Part model, mm, in its own coordinate system. A direction names the side the tool comes from. Round coordinates to 2 decimals unless told otherwise and drop trailing zeros. Loops run counter-clockwise (first coordinate to the right, second up) from the corner with the lowest first, then second, coordinate; pieces in that order, holes last. Notation, with made-up numbers: M 76.5,84 L 109.5,84 A12 ccw 109.5,102 Z; hole C 74.5,56.5 d2. An arc over 180 degrees is marked long. Put each result on its own line as item: value. Start each with the question number.
```python
from build123d import *

# Parameters (mm, degrees)
GBT706_2008_16A_1_DEPTH = 1637
CUT_EXTRUDE_1_DEPTH     = 837.367891541
CUT_EXTRUDE_2_DEPTH     = 837.367891541
SKETCH_4_W              = 56.5
SKETCH_4_H              = 56.5
CUT_EXTRUDE_3_DEPTH     = 835.965313439
SKETCH_5_W              = 56.5
SKETCH_5_H              = 56.5
CUT_EXTRUDE_4_DEPTH     = 835.965313439
CUT_EXTRUDE_5_REACH     = 838.368


with BuildPart() as part:
    # Sketch12 → Gbt706-2008 热轧槽钢 16A(1) (new body)
    with BuildSketch(Plane.YZ.offset(-818.5)):
        with BuildLine():
            Line((63, 160), (0, 160))
            Line((0, 160), (0, 0))
            Line((0, 0), (63, 0))
            Line((63, 0), (63, 2.528785132))
            ThreePointArc((63, 2.528785132), (61.715724127, 5.874438164), (58.522642316, 7.501394609))
            Line((58.522642316, 7.501394609), (15.454715367, 12.028016136))
            ThreePointArc((15.454715367, 12.028016136), (9.068551745, 15.281929026), (6.5, 21.973235089))
            Line((6.5, 21.973235089), (6.5, 138.026764911))
            ThreePointArc((6.5, 138.026764911), (9.068551745, 144.718070974), (15.454715367, 147.971983864))
            Line((15.454715367, 147.971983864), (58.522642316, 152.498605391))
            ThreePointArc((58.522642316, 152.498605391), (61.715724127, 154.125561836), (63, 157.471214868))
            Line((63, 157.471214868), (63, 160))
        make_face()
    extrude(amount=GBT706_2008_16A_1_DEPTH)

    # 草图2 → 切除-拉伸1 (cut, through all)
    with BuildSketch(Plane.XZ):
        Polygon((762, -5), (762, 7.501394609), (766.477357684, 7.501394609), (809.545284633, 12.028016136), (818.5, 21.973235089), (818.5, 138.026764911), (809.545284633, 147.971983864), (766.477357684, 152.498605391), (762, 152.498605391), (762, 165), (828.5, 165), (828.5, -5), align=None)
    extrude(amount=-CUT_EXTRUDE_1_DEPTH, mode=Mode.SUBTRACT)

    # 草图3 → 切除-拉伸2 (cut, through all)
    with BuildSketch(Plane.XZ):
        Polygon((-762, 0), (-762, 7.501394609), (-766.477357684, 7.501394609), (-809.545284633, 12.028016136), (-818.5, 21.973235089), (-818.5, 138.026764911), (-809.545284633, 147.971983864), (-766.477357684, 152.498605391), (-762, 152.498605391), (-762, 165), (-838.5, 165), (-838.5, -5), (-762, -5), align=None)
    extrude(amount=-CUT_EXTRUDE_2_DEPTH, mode=Mode.SUBTRACT)

    # 草图4 → 切除-拉伸3 (cut, through all)
    with BuildSketch(Plane.XY.offset(152.498605391)):
        with Locations((790.25, 34.75)):
            Rectangle(SKETCH_4_W, SKETCH_4_H)
    extrude(amount=-CUT_EXTRUDE_3_DEPTH, mode=Mode.SUBTRACT)

    # 草图5 → 切除-拉伸4 (cut, through all)
    with BuildSketch(Plane.XY.offset(152.498605391)):
        with Locations((-790.25, 34.75)):
            Rectangle(SKETCH_5_W, SKETCH_5_H)
    extrude(amount=-CUT_EXTRUDE_4_DEPTH, mode=Mode.SUBTRACT)

    # 草图6 → 切除-拉伸5 (cut, up to next)
    with BuildSketch(Plane.XZ, mode=Mode.PRIVATE) as cut_extrude_5_sk1:
        with BuildLine():
            Line((-580, 20), (-720, 20))
            ThreePointArc((-720, 20), (-723.535533906, 21.464466094), (-725, 25))
            Line((-725, 25), (-725, 105))
            ThreePointArc((-725, 105), (-723.535533906, 108.535533906), (-720, 110))
            Line((-720, 110), (-580, 110))
            ThreePointArc((-580, 110), (-576.464466094, 108.535533906), (-575, 105))
            Line((-575, 105), (-575, 25))
            ThreePointArc((-575, 25), (-576.464466094, 21.464466094), (-580, 20))
        make_face()
    cut_extrude_5_tool1 = extrude(cut_extrude_5_sk1.sketch, amount=-CUT_EXTRUDE_5_REACH, mode=Mode.PRIVATE) & part.part
    # 草图6 → 切除-拉伸5 (cut, up to next)
    with BuildSketch(Plane.XZ, mode=Mode.PRIVATE) as cut_extrude_5_sk2:
        with BuildLine():
            Line((-375, 25), (-375, 105))
            ThreePointArc((-375, 105), (-376.464466094, 108.535533906), (-380, 110))
            Line((-380, 110), (-520, 110))
            ThreePointArc((-520, 110), (-523.535533906, 108.535533906), (-525, 105))
            Line((-525, 105), (-525, 25))
            ThreePointArc((-525, 25), (-523.535533906, 21.464466094), (-520, 20))
            Line((-520, 20), (-380, 20))
            ThreePointArc((-380, 20), (-376.464466094, 21.464466094), (-375, 25))
        make_face()
    cut_extrude_5_tool2 = extrude(cut_extrude_5_sk2.sketch, amount=-CUT_EXTRUDE_5_REACH, mode=Mode.PRIVATE) & part.part
    add(cut_extrude_5_tool1.solids().sort_by_distance((-650, 0, 65))[0], mode=Mode.SUBTRACT)
    add(cut_extrude_5_tool2.solids().sort_by_distance((-450, 0, 65))[0], mode=Mode.SUBTRACT)


solid = part.part
```
1. Cut at B-B, the plane x = -457.5. Give the cut face in (y, z), and give its area (3 significant figures).
2. Cut at C-C, the plane y = 29. Give the cut face in (x, z).
3. Drop flat-ended pins along their axis: pin 1 (2 mm diameter, centred on x = -765, y = 2, fed in from +Z); pin 2 (1.3 mm diameter, centred on x = 764, y = 4.5, fed in from -Z); pin 3 (6.5 mm diameter, centred on y = 28.5, z = 146.5, fed in from -X). Give the stop position or say it passes through.
4. Cut at D-D, the plane x = 609. Give the cut face in (y, z).
5. Wall check: L1, parallel to Z at x = -111, y = 56; L2, parallel to Z at x = -131.5, y = 17; L3, parallel to Y at x = 568.5, z = 111.5. Give the ranges that are in metal, low to high.
6. Cut at A-A, the plane z = 76. Give the cut face in (x, y).
7. Mould opens along Z. For faces 1 (the flat face through (-10.668, 36.687, 150.204)), 2 (the flat face through (-11, 32, 160)), 3 (the flat face through (-11, 0, 81)) say: released by +Z, released by -Z, zero draft, split by the parting line, or undercut.
8. Which spindle directions (+Z, -Z, +X, -X, +Y, -Y) get a long thin tool onto all of the face, cutting with end or side? Do faces 4 (the flat face through (-10.668, 37.29, 9.733)), 5 (the flat face through (-11, 31, 0)). Say none if no direction does.
Results list:
1. outline: M 0,0 L 63,0 L 63,2.53 A5 ccw 58.52,7.5 L 15.45,12.03 A10 cw 6.7,20 L 0,20 Z; M 0,110 L 6.5,110 L 6.5,138.03 A10 cw 15.45,147.97 L 58.52,152.5 A5 ccw 63,157.47 L 63,160 L 0,160 Z
1. area: 1,610 mm^2
2. outline: M -762,0 L 762,0 L 762,10.6 L -762,10.6 Z; M -762,149.4 L 762,149.4 L 762,160 L -762,160 Z
3. pin 1: stops at z = 152.5
3. pin 2: stops at z = 7.5
3. pin 3: stops at x = -762
4. outline: M 0,0 L 63,0 L 63,2.53 A5 ccw 58.52,7.5 L 15.45,12.03 A10 cw 6.5,21.97 L 6.5,138.03 A10 cw 15.45,147.97 L 58.52,152.5 A5 ccw 63,157.47 L 63,160 L 0,160 Z
5. L1: z = 0 to 7.77, 152.23 to 160
5. L2: z = 0 to 11.87, 148.13 to 160
5. L3: y = 0 to 6.5
6. outline: M -818.5,0 L -725,0 L -725,6.5 L -818.5,6.5 Z; M -575,0 L -525,0 L -525,6.5 L -575,6.5 Z; M -375,0 L 818.5,0 L 818.5,6.5 L -375,6.5 Z
7. face 1: undercut
7. face 2: released by +Z
7. face 3: zero draft
8. face 4: +X, -X, +Y
8. face 5: -Z, +X, -X, +Y, -Y
